```python
from build123d import *
from OCP.BRepFilletAPI import BRepFilletAPI_MakeChamfer

# Parameters (mm, degrees)
SKETCH1_R           = 8
BOSS_EXTRUDE1_DEPTH = 10
CUT_EXTRUDE1_DEPTH  = 5
SKETCH3_R           = 5
BOSS_EXTRUDE2_DEPTH = 50
CHAMFER1_SIZE       = 1.25
FILLET1_R           = 1.230769231
CHAMFER2_SIZE       = 2.305475504
CHAMFER2_SIZE2      = 3.993200709
FILLET2_R           = 0.1


with BuildPart() as part:
    # Sketch1 → Boss-Extrude1 (new body)
    with BuildSketch(Plane.XY):
        Circle(SKETCH1_R)
    extrude(amount=BOSS_EXTRUDE1_DEPTH)

    # Sketch2 → Cut-Extrude1 (cut)
    with BuildSketch(Plane.XY.offset(10)):
        Polygon((4, 2.309401077), (0, 4.618802154), (-4, 2.309401077), (-4, -2.309401077), (0, -4.618802154), (4, -2.309401077), align=None)
    extrude(amount=-CUT_EXTRUDE1_DEPTH, mode=Mode.SUBTRACT)

    # Sketch3 → Boss-Extrude2 (add)
    with BuildSketch(Plane(origin=(0, 0, 0), x_dir=(-1, 0, 0), z_dir=(0, 0, -1))):
        with Locations(Location((0, 0, 0), (0, 0, 180))):
            Circle(SKETCH3_R)
    extrude(amount=BOSS_EXTRUDE2_DEPTH)

    # Chamfer1
    chamfer1_edges = [part.edges().sort_by_distance(p)[0] for p in [
        (-5, 0, -50),
    ]]
    chamfer(chamfer1_edges, length=CHAMFER1_SIZE)

    # Fillet1
    fillet1_edges = [part.edges().sort_by_distance(p)[0] for p in [
        (-8, 0, 10),
    ]]
    fillet(fillet1_edges, radius=FILLET1_R)

    # Chamfer2: one chamfer whose edges measure the first distance from different faces: ONE call of the kernel's chamfer builder (chamfer() names one face for all edges)
    chamfer2_edges_1 = [part.edges().sort_by_distance(p)[0] for p in [
        (-2, 3.464101615, 5),
    ]]
    chamfer2_side_1 = [part.faces().sort_by_distance(p)[0] for p in [
        (-2, 3.464101615, 7.5),
    ]]
    chamfer2_edges_2 = [part.edges().sort_by_distance(p)[0] for p in [
        (2, 3.464101615, 5),
    ]]
    chamfer2_side_2 = [part.faces().sort_by_distance(p)[0] for p in [
        (2, 3.464101615, 7.5),
    ]]
    chamfer2_edges_3 = [part.edges().sort_by_distance(p)[0] for p in [
        (4, 0, 5),
    ]]
    chamfer2_side_3 = [part.faces().sort_by_distance(p)[0] for p in [
        (4, 0, 7.5),
    ]]
    chamfer2_edges_4 = [part.edges().sort_by_distance(p)[0] for p in [
        (2, -3.464101615, 5),
    ]]
    chamfer2_side_4 = [part.faces().sort_by_distance(p)[0] for p in [
        (2, -3.464101615, 7.5),
    ]]
    chamfer2_edges_5 = [part.edges().sort_by_distance(p)[0] for p in [
        (-2, -3.464101615, 5),
    ]]
    chamfer2_side_5 = [part.faces().sort_by_distance(p)[0] for p in [
        (-2, -3.464101615, 7.5),
    ]]
    chamfer2_edges_6 = [part.edges().sort_by_distance(p)[0] for p in [
        (-4, 0, 5),
    ]]
    chamfer2_side_6 = [part.faces().sort_by_distance(p)[0] for p in [
        (-4, 0, 7.5),
    ]]
    chamfer2 = BRepFilletAPI_MakeChamfer(part.part.solid().wrapped)
    for e in chamfer2_edges_1:
        chamfer2.Add(CHAMFER2_SIZE, CHAMFER2_SIZE2, e.wrapped, chamfer2_side_1[0].wrapped)  # the first distance lies on this face
    for e in chamfer2_edges_2:
        chamfer2.Add(CHAMFER2_SIZE, CHAMFER2_SIZE2, e.wrapped, chamfer2_side_2[0].wrapped)  # the first distance lies on this face
    for e in chamfer2_edges_3:
        chamfer2.Add(CHAMFER2_SIZE, CHAMFER2_SIZE2, e.wrapped, chamfer2_side_3[0].wrapped)  # the first distance lies on this face
    for e in chamfer2_edges_4:
        chamfer2.Add(CHAMFER2_SIZE, CHAMFER2_SIZE2, e.wrapped, chamfer2_side_4[0].wrapped)  # the first distance lies on this face
    for e in chamfer2_edges_5:
        chamfer2.Add(CHAMFER2_SIZE, CHAMFER2_SIZE2, e.wrapped, chamfer2_side_5[0].wrapped)  # the first distance lies on this face
    for e in chamfer2_edges_6:
        chamfer2.Add(CHAMFER2_SIZE, CHAMFER2_SIZE2, e.wrapped, chamfer2_side_6[0].wrapped)  # the first distance lies on this face
    add(Compound.cast(chamfer2.Shape()), mode=Mode.REPLACE)

    # Fillet2
    fillet2_edges = [part.edges().sort_by_distance(p)[0] for p in [
        (-5, 0, 0),
    ]]
    fillet(fillet2_edges, radius=FILLET2_R)


solid = part.part
```
Geometry: final body of the model. Coordinates: model frame, mm. A direction names the side the tool comes from. Give positions to 0.01 mm unless a question says otherwise; leave off trailing zeros. Order: outer loops, then holes, each group sorted by start corner. A loop starts at its lowest first (then second) coordinate and runs counter-clockwise, first axis right, second up. Notation, with made-up numbers: M -26,-23.75 L 17,-23.75 A34 ccw 17,15.25 Z; hole C -1.5,-16 d10. An arc over 180 degrees is marked long. Answer as CSV lines item,"result". Start each with the question number.
1) Set-up query: faces 1 (the flat face through (0, 0, -50)), 2 (the flat face through (1.18, -2.11, 6.39)). Return all of +Z, -Z, +X, -X, +Y, -Y with unobstructed straight access to the full face (end or side cutting, diameter ignored); none if empty.
2) Line query: line 1 (Z direction, x = -1.5, y = -6.5); line 2 (Y direction, x = -1, z = 7); line 3 (Y direction, x = -3, z = -41). Output: solid intervals per line, ascending. Write a range as from..to.
3) Mould query, pull axis Y, two halves, no side actions, for faces 3 (the cylindrical face through (-5, 0, -24)), 4 (the flat face through (-1.18, 2.11, 6.39)), 5 (the flat face through (5, -2, 0)). Classes: +Y half, -Y half, draft (parallel to the pull), parting line (faces both ways), or undercut.
4) Cut plane A-A (z = -4). Output: boundary loops of the cut face in (x, y), then the cut area to 3 significant figures.
5) First-contact query: P1, Ø8, axis at x = -1.5, z = -36, coming from the -Y side; P2, Ø5, axis at y = 4.5, z = 3.5, coming from the -X side; P3, Ø2, axis at y = 0.5, z = 8.5, coming from the -X side; P4, Ø1, axis at x = 4, z = -28.5, coming from the -Y side. Flat tips, straight axial feed; report the tip coordinate or a pass-through.
Findings below:
1,face 1,"-Z, +X, -X, +Y, -Y"
1,face 2,"+Z"
2,line 1,"z = 0..10"
2,line 2,"y = -7.94..-3.43, 3.43..7.94"
2,line 3,"y = -4..4"
3,face 3,"parting line"
3,face 4,"undercut"
3,face 5,"draft"
4,outline,"C 0,0 d10"
4,area,"78.5 mm²"
5,P1,"stops at y = -5"
5,P2,"stops at x = -7.75"
5,P3,"stops at x = -8"
5,P4,"stops at y = -3.57"
